Input: part model. Units: mm. Frame: model coordinates. Coordinates: 2 decimals unless noted, no trailing zeros. Write each loop counter-clockwise with the first axis right and the second up, starting at its lowest first coordinate (ties: lowest second). Pieces come first, ordered by that corner, then holes.
1) Section query B-B (z = 0.9). Output: boundary loops of the cut face in (x, y), then the cut area to 3 significant figures.
2) Pin query (flat end, axial travel): pin 1 Ø4 at (x, y) = (-200, 200) entering from -Z. Return the tip coordinate at first contact, or that it passes through.
3) Section query C-C (x = 152). Output: boundary loops of the cut face in (y, z).
4) Line query: L1, parallel to Y at x = 200, z = 0.8; L2, parallel to X at y = -138, z = 0.25. Output: solid intervals per line, ascending.
5) Section query A-A (y = -117.5). Output: boundary loops of the cut face in (x, z).
from build123d import *

# Parameters (mm, degrees)
SKETCH_1_W            = 500
SKETCH_1_H            = 500
EXTRUDE_1_DEPTH       = 2
HOLE_WIZARD_7_0_7_1_D = 7
SKETCH_4_W            = 100
SKETCH_4_H            = 150
CUT_EXTRUDE_1_DEPTH   = 354.559047402


with BuildPart() as part:
    # 草图1 → 凸台-拉伸1 (new body)
    with BuildSketch(Plane.XY):
        Rectangle(SKETCH_1_W, SKETCH_1_H)
    extrude(amount=EXTRUDE_1_DEPTH)

    # Ø7.0 (7) 直径孔1 (through all)
    with Locations(Plane.XY.offset(2)):
        with Locations((-200, 200), (200, 200), (-200, -200), (200, -200)):
            Hole(HOLE_WIZARD_7_0_7_1_D / 2)

    # 草图4 → 切除-拉伸1 (cut, through all)
    with BuildSketch(Plane.XY.offset(2)):
        with Locations((130, -100)):
            Rectangle(SKETCH_4_W, SKETCH_4_H)
    extrude(amount=-CUT_EXTRUDE_1_DEPTH, mode=Mode.SUBTRACT)


solid = part.part
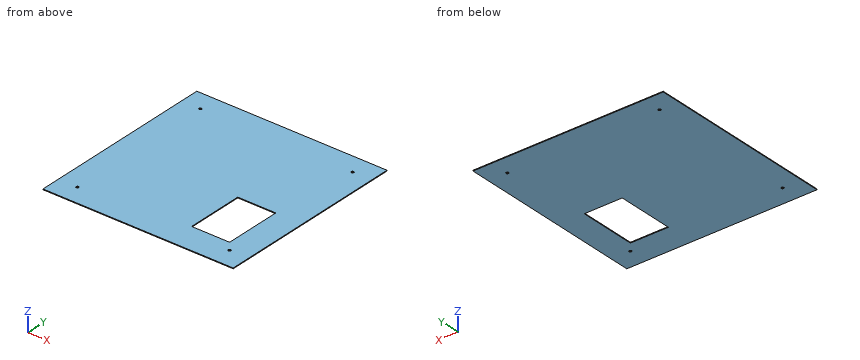
Answer:
1. outline: (-250, -250) - (250, -250) - (250, 250) - (-250, 250) - close; hole circle Ø7 at (-200, -200); hole circle Ø7 at (-200, 200); hole (80, -175) - (180, -175) - (180, -25) - (80, -25) - close; hole circle Ø7 at (200, -200); hole circle Ø7 at (200, 200)
1. area: 235,000 mm2
2. pin 1: passes through
3. outline: (-250, 0) - (-175, 0) - (-175, 2) - (-250, 2) - close; (-25, 0) - (250, 0) - (250, 2) - (-25, 2) - close
4. L1: y = -250 to -203.5, -196.5 to 196.5, 203.5 to 250
4. L2: x = -250 to 80, 180 to 250
5. outline: (-250, 0) - (80, 0) - (80, 2) - (-250, 2) - close; (180, 0) - (250, 0) - (250, 2) - (180, 2) - close
